For this review, take the finished solid that the model builds, in its own axes (mm). Face numbers are marked on the shaded views. Give positions to 0.01 mm unless a question says otherwise; leave off trailing zeros. Order: outer loops, then holes, each group sorted by start corner. A loop starts at its lowest first (then second) coordinate and runs counter-clockwise, first axis right, second up.
from build123d import *

# Parameters (mm, degrees)
SKETCH1_W                  = 85
SKETCH1_H                  = 16
EXTRUDE1_DEPTH             = 6
F_8_2_8_2_DIAMETER_HOLE1_D = 8.2
CHAMFER1_SIZE              = 2
SKETCH5_W                  = 15
SKETCH5_H                  = 16
CUT_EXTRUDE1_DEPTH         = 2


with BuildPart() as part:
    # Sketch1 → Extrude1 (new body)
    with BuildSketch(Plane(origin=(0, 0, 0), x_dir=(0, 0, -1), z_dir=(1, 0, 0))):
        with Locations((42.5, -8)):
            Rectangle(SKETCH1_W, SKETCH1_H)
        with BuildLine():
            Line((22, -4.75), (77, -4.75))
            ThreePointArc((77, -4.75), (80.25, -8), (77, -11.25))
            Line((77, -11.25), (22, -11.25))
            ThreePointArc((22, -11.25), (18.75, -8), (22, -4.75))
        make_face(mode=Mode.SUBTRACT)
    extrude(amount=EXTRUDE1_DEPTH)

    # Ø8.2 (8.2) Diameter Hole1 (through all)
    with Locations(Plane(origin=(6, 0, 0), x_dir=(0, 0, -1), z_dir=(1, 0, 0))):
        with Locations((7, -8)):
            Hole(F_8_2_8_2_DIAMETER_HOLE1_D / 2)

    # Chamfer1
    chamfer1_edges = [part.edges().sort_by_distance(p)[0] for p in [
        (3, 0, 0),
        (3, 0, -85),
        (3, -16, -85),
        (3, -16, 0),
    ]]
    chamfer(chamfer1_edges, length=CHAMFER1_SIZE)

    # Sketch5 → Cut-Extrude1 (cut)
    with BuildSketch(Plane(origin=(6, 0, 0), x_dir=(0, 0, -1), z_dir=(1, 0, 0))):
        with Locations((7.5, -8)):
            Rectangle(SKETCH5_W, SKETCH5_H)
    extrude(amount=-CUT_EXTRUDE1_DEPTH, mode=Mode.SUBTRACT)


solid = part.part
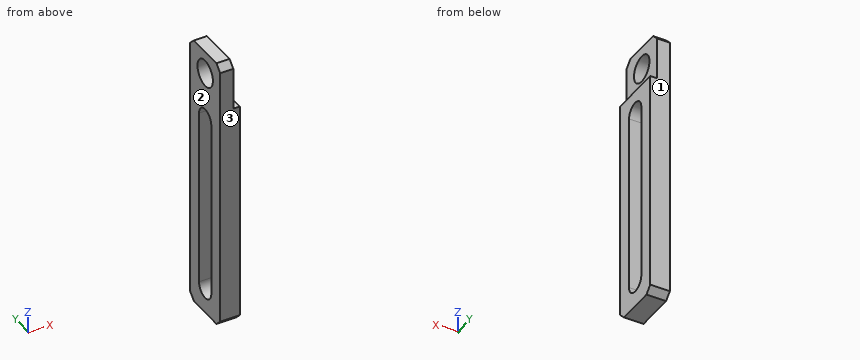
1) To check wall thickness, follow line 1 (Y direction, x = 3.2, z = -56); line 2 (Z direction, x = 2.7, y = -10); line 3 (Y direction, x = 1.6, z = -7). State the ranges of each line that lie inside material, in increasing order.
Answer sheet:
line 1: y = -16 to -11.25, -4.75 to 0
line 2: z = -85 to -79.56, -19.44 to -10.58, -3.42 to 0
line 3: y = -16 to -12.1, -3.9 to 0
2) We need section A-A on y = -8. Give the boundary of the cut face in (x, z).
Answer sheet:
outline: (0, -85) - (6, -85) - (6, -80.25) - (0, -80.25) - close; (0, -18.75) - (6, -18.75) - (6, -15) - (4, -15) - (4, -11.1) - (0, -11.1) - close; (0, -2.9) - (4, -2.9) - (4, 0) - (0, 0) - close
3) We need section B-B on x = 3. Give the boundary of the cut face in (y, z).
Answer sheet:
outline: (-16, -83) - (-14, -85) - (-2, -85) - (0, -83) - (0, -2) - (-2, 0) - (-14, 0) - (-16, -2) - close; hole circle Ø8.2 at (-8, -7); hole (-11.25, -77) arc R3.25 ccw to (-4.75, -77) - (-4.75, -22) arc R3.25 ccw to (-11.25, -22) - close
4) We need section C-C on z = -45. Give the boundary of the cut face in (x, y), then the cut area to 3 significant figures.
Answer sheet:
outline: (0, -16) - (6, -16) - (6, -11.25) - (0, -11.25) - close; (0, -4.75) - (6, -4.75) - (6, 0) - (0, 0) - close
area: 57.0 mm2
5) Draft analysis for pull direction Y (two halves, no side actions). For the marked faces 1, 2 and 3, state which applies: +Y half, -Y half, draft (parallel to the pull), parting line (faces both ways), or undercut.
Answer sheet:
face 1: +Y half
face 2: draft
face 3: -Y half
6) Clearance check with flat-ended pins moving along their axes: pin 1 (4.5 mm diameter, centred on y = -11, z = -9, fed in from +X); pin 2 (1 mm diameter, centred on x = 5.5, y = -11.5, fed in from +Z); pin 3 (7.5 mm diameter, centred on y = -8, z = -7, fed in from -X). State where each tip first meets the part, or that it passes through.
Answer sheet:
pin 1: stops at x = 4
pin 2: stops at z = -15
pin 3: passes through
